Can you work these out from the model? Positions are in its coordinate system, mm. Coordinates: 2 decimals unless noted, no trailing zeros. Order: outer loops, then holes, each group sorted by start corner. A loop starts at its lowest first (then second) coordinate and runs counter-clockwise, first axis right, second up. Notation, with made-up numbers: (66.5, 33) -> (98.5, 33) arc R27 ccw to (98.5, 65) -> close; hole circle Ø8 at (0, 20). An arc over 180 degrees is marked (long way). Answer in a Markdown table with one row per item.
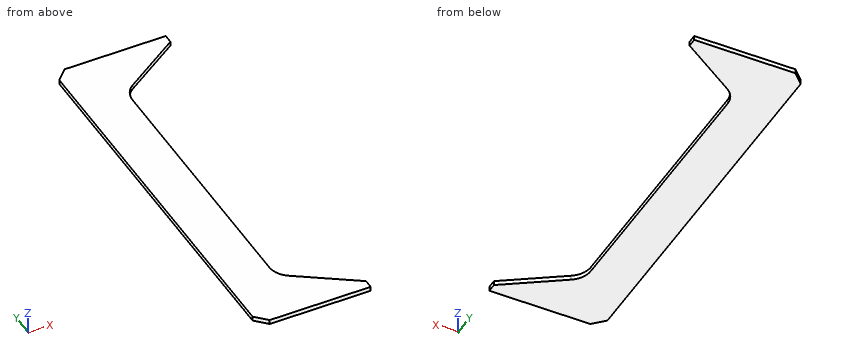
```python
from build123d import *

# Parameters (mm, degrees)
SKETCH1_W           = 150
SKETCH1_H           = 20
SKETCH1_W_2         = 100
BOSS_EXTRUDE1_DEPTH = 10
FILLET1_R           = 50
CHAMFER1_SIZE       = 25


with BuildPart() as part:
    # Sketch1 → Boss-Extrude1 (new body)
    with BuildSketch(Plane.XY):
        Polygon((200, 420), (50, 420), (50, 320), align=None)
        with Locations((125, 430)):
            Rectangle(SKETCH1_W, SKETCH1_H)
        Polygon((-50, 420), (-50, -420), (50, -420), (50, -320), (50, 320), (50, 420), align=None)
        Polygon((50, -320), (50, -420), (200, -420), align=None)
        with Locations((125, -430)):
            Rectangle(SKETCH1_W, SKETCH1_H)
        with Locations((0, -430)):
            Rectangle(SKETCH1_W_2, SKETCH1_H)
        with Locations((0, 430)):
            Rectangle(SKETCH1_W_2, SKETCH1_H)
    extrude(amount=BOSS_EXTRUDE1_DEPTH)

    # Fillet1
    fillet1_edges = [part.edges().sort_by_distance(p)[0] for p in [
        (50, 320, 5),
        (50, -320, 5),
    ]]
    fillet(fillet1_edges, radius=FILLET1_R)

    # Chamfer1
    chamfer1_edges = [part.edges().sort_by_distance(p)[0] for p in [
        (-50, -440, 5),
        (-50, 440, 5),
    ]]
    chamfer(chamfer1_edges, length=CHAMFER1_SIZE)


solid = part.part
```
(1) Suppose I cut it at C-C (y = -22). Please give me the cut outline in (x, z), and give its area (3 significant figures).
Response values:
| item | result |
|---|---|
| outline | (-50, 0) -> (50, 0) -> (50, 10) -> (-50, 10) -> close |
| area | 1,000 mm2 |
(2) Suppose I cut it at D-D (x = 178). Please give me the cut outline in (y, z), and give its area (3 significant figures).
Response values:
| item | result |
|---|---|
| outline | (-440, 0) -> (-405.33, 0) -> (-405.33, 10) -> (-440, 10) -> close; (405.33, 0) -> (440, 0) -> (440, 10) -> (405.33, 10) -> close |
| area | 693 mm2 |
(3) Suppose I cut it at B-B (z = 2.5). Please give me the cut outline in (x, y) (3 decimals), and give its area (3 significant figures).
Response values:
| item | result |
|---|---|
| outline | (-50, -415) -> (-25, -440) -> (200, -440) -> (200, -420) -> (72.265, -334.843) arc R50 cw to (50, -293.241) -> (50, 293.241) arc R50 cw to (72.265, 334.843) -> (200, 420) -> (200, 440) -> (-25, 440) -> (-50, 415) -> close |
| area | 109,000 mm2 |
(4) I need wall thicknesses on line 1 (X direction, y = -189.5, z = 8.75); line 2 (Y direction, x = 184, z = 9.25); line 3 (Y direction, x = 76, z = 9.5). Which ranges of each line are inside material? Lowest first, please. Write a range as [from, to].
Response values:
| item | result |
|---|---|
| line 1 | [-50, 50] |
| line 2 | [-440, -409.33], [409.33, 440] |
| line 3 | [-440, -337.33], [337.33, 440] |
(5) Suppose I cut it at A-A (x = 143). Please give me the cut outline in (y, z).
Response values:
| item | result |
|---|---|
| outline | (-440, 0) -> (-382, 0) -> (-382, 10) -> (-440, 10) -> close; (382, 0) -> (440, 0) -> (440, 10) -> (382, 10) -> close |
(6) Will this pin go through, and if not, where does the flat tip stop? pin 1 Ø5 at (x, y) = (24, -200) entering from -Z.
Response values:
| item | result |
|---|---|
| pin 1 | z = 0 |
